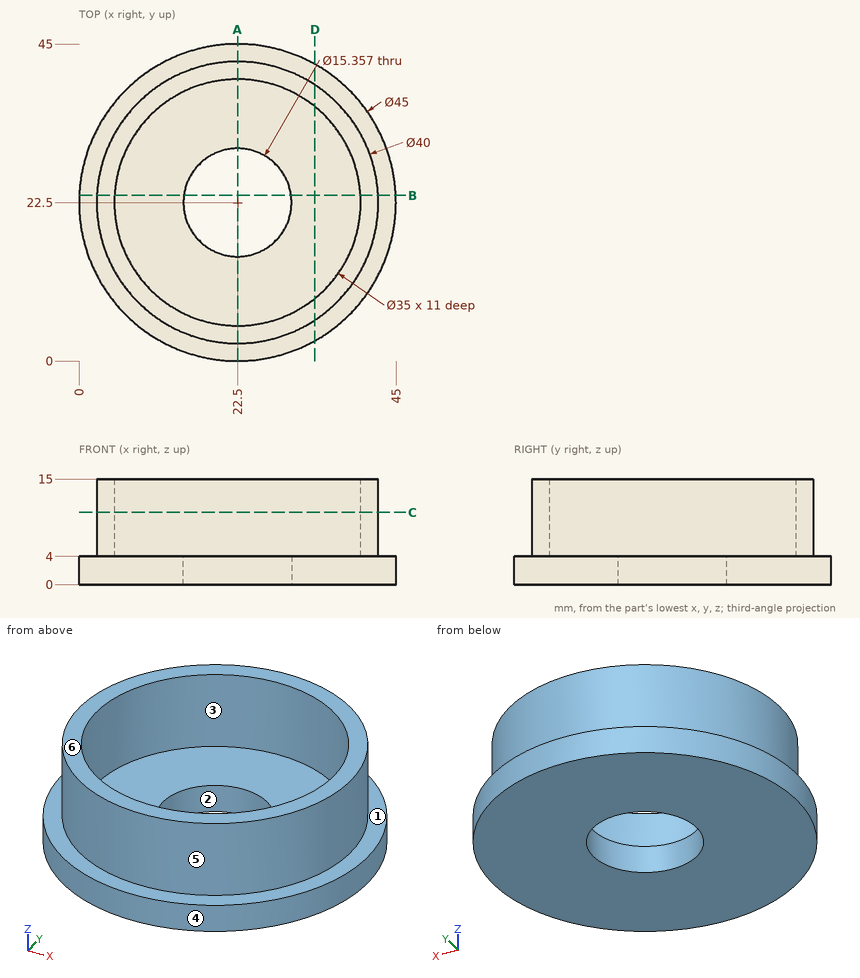
Here's the drawing with two shaded views (mm, measured from the low corner). I have some questions. A direction names the side the tool comes from. Give positions to 0.01 mm unless a question says otherwise; leave off trailing zeros. Order: outer loops, then holes, each group sorted by start corner. A loop starts at its lowest first (then second) coordinate and runs counter-clockwise, first axis right, second up. Notation, with made-up numbers: M 37.5,34 L 69.5,34 A21 ccw 69.5,49 Z; hole C -38.5,50 d2. An arc over 180 degrees is marked long. Answer as a JSON object with one key per item and string values. Group by question number.
1) Suppose I cut it at C-C, the plane z = 10.25. Write out the boundary of the cut face in (x, y).
2) Suppose I cut it at B-B, the plane y = 23.5. Write out the boundary of the cut face in (x, z) (1 decimal).
3) Suppose I cut it at D-D, the plane x = 33.5. Write out the boundary of the cut face in (y, z).
4) Please list where these lines run through material, in increasing order: L1, parallel to Y at x = 22.5, z = 7.75; L2, parallel to Y at x = 22.5, z = 2.4; L3, parallel to Z at x = 28, y = 32.5. Write a range as [from, to].
5) On a 3-axis mill with a long thin cutter (end or side, diameter ignored), from which of +Z, -Z, +X, -X, +Y, -Y can I reach the whole of each face in a straight line? I mean the marked faces 5 and 6. Say none if no direction works.
6) Suppose I cut it at A-A, the plane x = 22.5. Write out the boundary of the cut face in (y, z).
7) We'd pull the mould along Y, two halves only. Please class the marked faces 1, 2, 3 and 4: pulls with the +Y half, pulls with the -Y half, needs draft (parallel to the pull), parting line crosses it, or undercut.
8) I'm going to push flat-ended pins straight in: pin 1 Ø5 at (y, z) = (10, 1.5) entering from -X (1 decimal); pin 2 Ø2 at (x, z) = (32, 8) entering from -Y; pin 3 Ø4 at (y, z) = (6.5, 7) entering from -X. Where does each tip first touch, or does it pass through?
Results found:
{
 "1": {"outline": "C 22.5,22.5 d40; hole C 22.5,22.5 d35"},
 "2": {"outline": "M 0,0 L 14.9,0 L 14.9,4 L 5,4 L 5,15 L 2.5,15 L 2.5,4 L 0,4 Z; M 30.1,0 L 45,0 L 45,4 L 42.5,4 L 42.5,15 L 40,15 L 40,4 L 30.1,4 Z"},
 "3": {"outline": "M 2.87,0 L 42.13,0 L 42.13,4 L 39.2,4 L 39.2,15 L 36.11,15 L 36.11,4 L 8.89,4 L 8.89,15 L 5.8,15 L 5.8,4 L 2.87,4 Z"},
 "4": {"L1": "[2.5, 5], [40, 42.5]", "L2": "[0, 14.82], [30.18, 45]", "L3": "[0, 4]"},
 "5": {"face 5": "+Z", "face 6": "+Z, +X, -X, +Y, -Y"},
 "6": {"outline": "M 0,0 L 14.82,0 L 14.82,4 L 5,4 L 5,15 L 2.5,15 L 2.5,4 L 0,4 Z; M 30.18,0 L 45,0 L 45,4 L 42.5,4 L 42.5,15 L 40,15 L 40,4 L 30.18,4 Z"},
 "7": {"face 1": "needs draft", "face 2": "undercut", "face 3": "undercut", "face 4": "parting line crosses it"},
 "8": {"pin 1": "x = 2.3", "pin 2": "y = 4.4", "pin 3": "x = 8.22"}
}
